```python
from build123d import *

# Parameters (mm, degrees)
SKETCH1_W             = 38
SKETCH1_H             = 75
BOSS_EXTRUDE1_DEPTH   = 6
M8_TAPPED_HOLE1_D     = 6.8
M8_TAPPED_HOLE2_D     = 6.8
M6_TAPPED_HOLE1_D     = 5
M6_TAPPED_HOLE1_DEPTH = 12
CHAMFER1_SIZE         = 1


with BuildPart() as part:
    # Sketch1 → Boss-Extrude1 (new, symmetric)
    with BuildSketch(Plane.XY):
        Rectangle(SKETCH1_W, SKETCH1_H)
    extrude(amount=BOSS_EXTRUDE1_DEPTH, both=True)

    # M8 Tapped Hole1 (through all)
    with Locations(Plane.XY.offset(6)):
        with Locations((-10, 26.5)):
            Hole(M8_TAPPED_HOLE1_D / 2)

    # M8 Tapped Hole2 (through all)
    with Locations(Plane.XY.offset(6)):
        with Locations((10, 26.5)):
            Hole(M8_TAPPED_HOLE2_D / 2)

    # M6 Tapped Hole1
    with Locations(Plane(origin=(0, -37.5, 0), x_dir=(-1, 0, 0), z_dir=(0, -1, 0))):
        with Locations((10, 0), (-10, 0)):
            Hole(M6_TAPPED_HOLE1_D / 2, depth=M6_TAPPED_HOLE1_DEPTH)

    # Chamfer1
    chamfer1_edges = [part.edges().sort_by_distance(p)[0] for p in [
        (19, -37.5, 0),
        (-19, -37.5, 0),
        (-19, 37.5, 0),
        (19, 37.5, 0),
    ]]
    chamfer(chamfer1_edges, length=CHAMFER1_SIZE)


solid = part.part
```
Work out the finished part from the listing and answer in its coordinate system (mm). A direction names the side the tool comes from. Give positions to 0.01 mm unless a question says otherwise; leave off trailing zeros. Loops run counter-clockwise (first coordinate to the right, second up) from the corner with the lowest first, then second, coordinate; pieces in that order, holes last. Notation, with made-up numbers: (64, 76.25) - (95, 76.25) arc R32 ccw to (95, 112.25) - close; hole circle Ø11 at (-38.75, -17). An arc over 180 degrees is marked (long way). Use CSV: the item, a comma, the result in double quotes. Start each with the question number.
(1) A tool of negligible diameter and unlimited length cuts with its end or side. For faces 4 (the face through (7.5, -31.4, -0.1)), 5 (the face through (0, -37.5, 0)), from which of +Z, -Z, +X, -X, +Y, -Y can it reach the whole face along a straight path? Write none if from no direction.
(2) Find section A-A, the plane y = 26.5. Determine the outline of the cut face in (x, z), plus the area to 3 significant figures.
(3) Find section B-B, the plane x = -10. Determine the outline of the cut face in (y, z), plus the area to 3 significant figures.
(4) Determine the mould class of faces 1 (the face through (-13.243, 27.521, -0.084)), 2 (the face through (-10, -25.5, 0)), 3 (the face through (0, 1, 6)) for opening direction Y: released by +Y, released by -Y, zero draft, split by the parting line, or undercut.
(5) Find section C-C, the plane z = 0. Determine the outline of the cut face in (x, y).
(6) Find the intervals of material crossed by L1, parallel to Y at x = -10, z = 1.25; L2, parallel to X at y = 27, z = -3; L3, parallel to Z at x = 10, y = -30.5, in increasing order.
(7) Find section D-D, the plane y = -26.5. Determine the outline of the cut face in (x, z).
(8) This flat-tipped pin is pushed along its axis until it touches: pin 1 (4.5 mm diameter, centred on x = 10, z = 0, fed in from -Y). Where does it stop, or does it pass through?
Results found:
1,face 4,"-Y"
1,face 5,"+Z, -Z, +X, -X, -Y"
2,outline,"(-19, -6) - (-13.4, -6) - (-13.4, 6) - (-19, 6) - close; (-6.6, -6) - (6.6, -6) - (6.6, 6) - (-6.6, 6) - close; (13.4, -6) - (19, -6) - (19, 6) - (13.4, 6) - close"
2,area,"293 mm^2"
3,outline,"(-37.5, -6) - (23.1, -6) - (23.1, 6) - (-37.5, 6) - (-37.5, 2.5) - (-25.5, 2.5) - (-25.5, -2.5) - (-37.5, -2.5) - close; (29.9, -6) - (37.5, -6) - (37.5, 6) - (29.9, 6) - close"
3,area,"758 mm^2"
4,face 1,"undercut"
4,face 2,"released by -Y"
4,face 3,"zero draft"
5,outline,"(-19, -36.5) - (-18, -37.5) - (-12.5, -37.5) - (-12.5, -25.5) - (-7.5, -25.5) - (-7.5, -37.5) - (7.5, -37.5) - (7.5, -25.5) - (12.5, -25.5) - (12.5, -37.5) - (18, -37.5) - (19, -36.5) - (19, 36.5) - (18, 37.5) - (-18, 37.5) - (-19, 36.5) - close; hole circle Ø6.8 at (-10, 26.5); hole circle Ø6.8 at (10, 26.5)"
6,L1,"-25.5 to 23.1, 29.9 to 37.5"
6,L2,"-19 to -13.36, -6.64 to 6.64, 13.36 to 19"
6,L3,"-6 to -2.5, 2.5 to 6"
7,outline,"(-19, -6) - (19, -6) - (19, 6) - (-19, 6) - close; hole circle Ø5 at (-10, 0); hole circle Ø5 at (10, 0)"
8,pin 1,"y = -25.5"
